For this review, take the finished solid that the model builds, in its own axes (mm). Face numbers are marked on the shaded views. A direction names the side the tool comes from. Coordinates: 2 decimals unless noted, no trailing zeros. Loops run counter-clockwise (first coordinate to the right, second up) from the corner with the lowest first, then second, coordinate; pieces in that order, holes last. Notation, with made-up numbers: (23.25, -38) -> (50.25, -38) arc R15 ccw to (50.25, -32) -> close; hole circle Ø7 at (-15, -35). An arc over 180 degrees is marked (long way). Use a Markdown table: item, result.
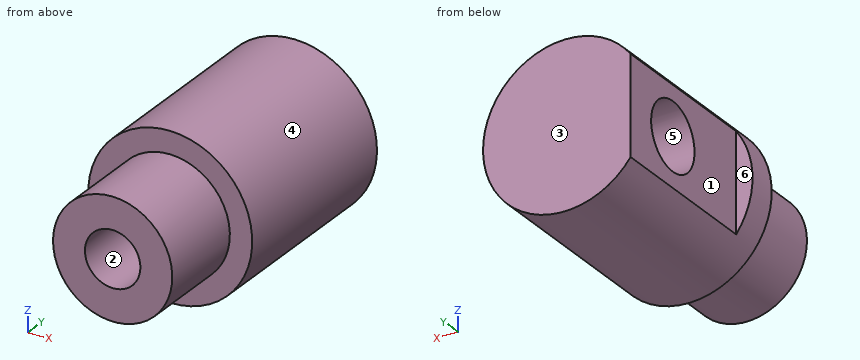
from build123d import *

# Parameters (mm, degrees)
SKETCH1_R           = 20
BOSS_EXTRUDE1_DEPTH = 30
SKETCH2_R           = 27.5
BOSS_EXTRUDE2_DEPTH = 65
CUT_EXTRUDE1_START  = -22
SKETCH3_W           = 35
SKETCH3_H           = 55
CUT_EXTRUDE1_DEPTH  = 65
SKETCH4_R           = 11.3
CUT_EXTRUDE2_DEPTH  = 40
SKETCH5_R           = 9.3
CUT_EXTRUDE3_DEPTH  = 74


with BuildPart() as part:
    # Sketch1 → Boss-Extrude1 (new body)
    with BuildSketch(Plane(origin=(0, 0, 0), x_dir=(1, 0, 0), z_dir=(0, 1, 0))):
        with Locations(Location((0, 0, 0), (0, 0, 270))):
            Circle(SKETCH1_R)
    extrude(amount=BOSS_EXTRUDE1_DEPTH)

    # Sketch2 → Boss-Extrude2 (add)
    with BuildSketch(Plane(origin=(0, 30, 0), x_dir=(1, 0, 0), z_dir=(0, 1, 0))):
        with Locations(Location((0, 0, 0), (0, 0, 270))):
            Circle(SKETCH2_R)
    extrude(amount=BOSS_EXTRUDE2_DEPTH)

    # Sketch3 → Cut-Extrude1 (cut)
    with BuildSketch(Plane(origin=(0, 0, 0), x_dir=(0, 0, -1), z_dir=(1, 0, 0)).offset(CUT_EXTRUDE1_START)):
        with Locations((0, 67.5)):
            Rectangle(SKETCH3_W, SKETCH3_H)
    extrude(amount=-CUT_EXTRUDE1_DEPTH, mode=Mode.SUBTRACT)

    # Sketch4 → Cut-Extrude2 (cut)
    with BuildSketch(Plane.ZY.offset(22)):
        with Locations((0, 73)):
            Circle(SKETCH4_R)
    extrude(amount=-CUT_EXTRUDE2_DEPTH, mode=Mode.SUBTRACT)

    # Sketch5 → Cut-Extrude3 (cut)
    with BuildSketch(Plane.XZ):
        with Locations(Location((0, 0, 0), (0, 0, 270))):
            Circle(SKETCH5_R)
    extrude(amount=-CUT_EXTRUDE3_DEPTH, mode=Mode.SUBTRACT)


solid = part.part
(1) Take a section at C-C on y = 10. Write out the cut boundary in (x, z), plus the area to 3 significant figures.
Found:
| item | result |
|---|---|
| outline | circle Ø40 at (0, 0); hole circle Ø18.6 at (0, 0) |
| area | 985 mm^2 |
(2) Take a section at A-A on z = 0. Write out the cut boundary in (x, y).
Found:
| item | result |
|---|---|
| outline | (-27.5, 30) -> (-20, 30) -> (-20, 0) -> (-9.3, 0) -> (-9.3, 61.7) -> (-22, 61.7) -> (-22, 40) -> (-27.5, 40) -> close; (-22, 84.3) -> (18, 84.3) -> (18, 61.7) -> (9.3, 61.7) -> (9.3, 0) -> (20, 0) -> (20, 30) -> (27.5, 30) -> (27.5, 95) -> (-22, 95) -> close |
(3) Take a section at D-D on z = 15. Write out the cut boundary in (x, y).
Found:
| item | result |
|---|---|
| outline | (-23.05, 30) -> (-13.23, 30) -> (-13.23, 0) -> (13.23, 0) -> (13.23, 30) -> (23.05, 30) -> (23.05, 95) -> (-22, 95) -> (-22, 40) -> (-23.05, 40) -> close |
(4) Mouldability with a two-part tool opening along Z and no side actions: class the marked faces 4, 5 and 6 as pulls with the +Z half, pulls with the -Z half, needs draft (parallel to the pull), parting line crosses it, or undercut.
Found:
| item | result |
|---|---|
| face 4 | parting line crosses it |
| face 5 | undercut |
| face 6 | needs draft |
(5) For line 1 along Z through (x, y) = (0, 34); line 2 along X through (y, z) = (25, 0); line 3 along Y through (x, z) = (-23, -11), list the stretches that pass through material, from the lowest coordinate up.
Found:
| item | result |
|---|---|
| line 1 | z = -27.5 to -9.3, 9.3 to 27.5 |
| line 2 | x = -20 to -9.3, 9.3 to 20 |
| line 3 | y = 30 to 40 |
(6) For the marked faces 1, 2 and 3, list the 3-axis set-ups (+Z, -Z, +X, -X, +Y, -Y) from which the entire face can be reached by the end or side of a thin tool; tool diameter is ignored.
Found:
| item | result |
|---|---|
| face 1 | +Z, -Z, -X, +Y |
| face 2 | -Y |
| face 3 | +Z, -Z, +X, -X, +Y |
(7) For pin 1 Ø2 at (x, z) = (16, -21) entering from -Y; pin 2 Ø5 at (y, z) = (41.5, -17) entering from +X; pin 3 Ø16.5 at (x, z) = (0, 0) entering from -Y, all flat-tipped, find the tip position at first contact; note any pin that passes through.
Found:
| item | result |
|---|---|
| pin 1 | stops at y = 30 |
| pin 2 | stops at x = 23.37 |
| pin 3 | stops at y = 80.72 |
(8) Take a section at B-B on x = 0. Write out the cut boundary in (y, z), plus the area to 3 significant figures.
Found:
| item | result |
|---|---|
| outline | (0, -20) -> (30, -20) -> (30, -27.5) -> (95, -27.5) -> (95, 27.5) -> (30, 27.5) -> (30, 20) -> (0, 20) -> (0, 9.3) -> (66.58, 9.3) arc R11.3 cw (long way) to (66.58, -9.3) -> (0, -9.3) -> close |
| area | 3,200 mm^2 |
